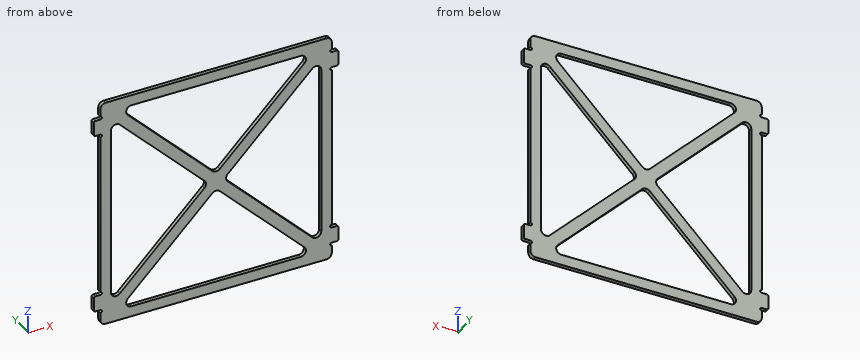
```python
from build123d import *

# Parameters (mm, degrees)
EXTRUDE_1_DEPTH = 1.5
FILLET_1_R      = 0.5
FILLET_2_R      = 2


with BuildPart() as part:
    # 草图1 → 凸台-拉伸1 (new body)
    with BuildSketch(Plane(origin=(0, 0, 0), x_dir=(1, 0, 0), z_dir=(0, 1, 0))):
        with BuildLine():
            Line((44.1, 44.1), (-44.1, 44.1))
            Line((-44.1, 44.1), (-44.1, 39.2))
            ThreePointArc((-44.1, 39.2), (-43.5, 38.6), (-44.1, 38))
            Line((-44.1, 38), (-46.6, 38))
            Line((-46.6, 38), (-46.6, 32))
            Line((-46.6, 32), (-44.1, 32))
            ThreePointArc((-44.1, 32), (-43.5, 31.4), (-44.1, 30.8))
            Line((-44.1, 30.8), (-44.1, -30.8))
            ThreePointArc((-44.1, -30.8), (-43.5, -31.4), (-44.1, -32))
            Line((-44.1, -32), (-46.6, -32))
            Line((-46.6, -32), (-46.6, -38))
            Line((-46.6, -38), (-44.1, -38))
            ThreePointArc((-44.1, -38), (-43.5, -38.6), (-44.1, -39.2))
            Line((-44.1, -39.2), (-44.1, -44.1))
            Line((-44.1, -44.1), (44.1, -44.1))
            Line((44.1, -44.1), (44.1, -39.2))
            ThreePointArc((44.1, -39.2), (43.5, -38.6), (44.1, -38))
            Line((44.1, -38), (46.6, -38))
            Line((46.6, -38), (46.6, -32))
            Line((46.6, -32), (44.1, -32))
            ThreePointArc((44.1, -32), (43.5, -31.4), (44.1, -30.8))
            Line((44.1, -30.8), (44.1, 30.8))
            ThreePointArc((44.1, 30.8), (43.5, 31.4), (44.1, 32))
            Line((44.1, 32), (46.6, 32))
            Line((46.6, 32), (46.6, 38))
            Line((46.6, 38), (44.1, 38))
            ThreePointArc((44.1, 38), (43.5, 38.6), (44.1, 39.2))
            Line((44.1, 39.2), (44.1, 44.1))
        make_face()
        Polygon((-37.1, 40.1), (37.1, 40.1), (0, 3), align=None, mode=Mode.SUBTRACT)
        Polygon((40.1, 37.1), (40.1, -37.1), (3, 0), align=None, mode=Mode.SUBTRACT)
        Polygon((37.1, -40.1), (-37.1, -40.1), (0, -3), align=None, mode=Mode.SUBTRACT)
        Polygon((-40.1, -37.1), (-40.1, 37.1), (-3, 0), align=None, mode=Mode.SUBTRACT)
    extrude(amount=EXTRUDE_1_DEPTH)

    # 圆角1
    fillet_1_edges = [part.edges().sort_by_distance(p)[0] for p in [
        (46.6, 0.75, -38),
        (46.6, 0.75, -32),
        (46.6, 0.75, 32),
        (46.6, 0.75, 38),
        (-46.6, 0.75, 38),
        (-46.6, 0.75, 32),
        (-46.6, 0.75, -32),
        (-46.6, 0.75, -38),
    ]]
    fillet(fillet_1_edges, radius=FILLET_1_R)

    # 圆角2
    fillet_2_edges = [part.edges().sort_by_distance(p)[0] for p in [
        (-44.1, 0.75, -44.1),
        (44.1, 0.75, -44.1),
        (44.1, 0.75, 44.1),
        (-44.1, 0.75, 44.1),
        (-40.1, 0.75, 37.1),
        (-3, 0.75, 0),
        (-40.1, 0.75, -37.1),
        (37.1, 0.75, 40.1),
        (0, 0.75, 3),
        (-37.1, 0.75, 40.1),
        (3, 0.75, 0),
        (40.1, 0.75, 37.1),
        (40.1, 0.75, -37.1),
        (0, 0.75, -3),
        (37.1, 0.75, -40.1),
        (-37.1, 0.75, -40.1),
    ]]
    fillet(fillet_2_edges, radius=FILLET_2_R)


solid = part.part
```
The model under review builds one solid part; all positions refer to its coordinate system, in mm. Round coordinates to 2 decimals unless told otherwise and drop trailing zeros. Loops run counter-clockwise (first coordinate to the right, second up) from the corner with the lowest first, then second, coordinate; pieces in that order, holes last.
1) Consider section C-C on y = 0.8. Give the number of separate pieces and of enclosed holes in the cut face, then the cut area to 3 significant figures.
Values follow:
separate pieces: 1
enclosed holes: 4
area: 2,370 mm2
2) Consider section A-A on x = -27.5. State the section outline as (y, z) points.
Values follow:
outline: (0, -44.1) - (1.5, -44.1) - (1.5, -40.1) - (0, -40.1) - close; (0, -30.5) - (1.5, -30.5) - (1.5, -24.5) - (0, -24.5) - close; (0, 24.5) - (1.5, 24.5) - (1.5, 30.5) - (0, 30.5) - close; (0, 40.1) - (1.5, 40.1) - (1.5, 44.1) - (0, 44.1) - close
3) Wall thickness on line 1 along Z through (x, y) = (35, 0.9); line 2 along X through (y, z) = (0.25, -30); line 3 along X through (y, z) = (0.8, -2): over which ranges is each line inside the solid? List them lowest first.
Values follow:
line 1: z = -44.1 to -32, 32 to 44.1
line 2: x = -44.1 to -40.1, -33 to -27, 27 to 33, 40.1 to 44.1
line 3: x = -44.1 to -40.1, -5 to 5, 40.1 to 44.1
4) Clearance check with flat-ended pins moving along their axes: P1, Ø0.8, axis at y = 0.5, z = 40.5, coming from the -X side; P2, Ø2, axis at x = 8.5, z = -15, coming from the -Y side; P3, Ø0.8, axis at x = 45, y = 0.5, coming from the +Z side; P4, Ø0.8, axis at x = -45, y = 0.5, coming from the -Z side. State where each tip first meets the part, or that it passes through.
Values follow:
P1: stops at x = -44.1
P2: passes through
P3: stops at z = 38
P4: stops at z = -38
5) Consider section B-B on z = 17.5. State the section outline as (x, y) points, then the cut area to 3 significant figures.
Values follow:
outline: (-44.1, 0) - (-40.1, 0) - (-40.1, 1.5) - (-44.1, 1.5) - close; (-20.5, 0) - (-14.5, 0) - (-14.5, 1.5) - (-20.5, 1.5) - close; (14.5, 0) - (20.5, 0) - (20.5, 1.5) - (14.5, 1.5) - close; (40.1, 0) - (44.1, 0) - (44.1, 1.5) - (40.1, 1.5) - close
area: 30.0 mm2
